```python
from build123d import *

# Parameters (mm, degrees)
EXTRUDE_1_DEPTH = 30


with BuildPart() as part:
    # 草图1 → 拉伸-薄壁1 (new body)
    with BuildSketch(Plane.XY):
        with BuildLine():
            Line((1246.5, -35.33), (-1246.5, -35.33))
            ThreePointArc((-1246.5, -35.33), (-1281.83, 0), (-1246.5, 35.33))
            Line((-1246.5, 35.33), (1246.5, 35.33))
            ThreePointArc((1246.5, 35.33), (1281.83, 0), (1246.5, -35.33))
        make_face()
        with BuildLine():
            Line((1246.5, -30.83), (-1246.5, -30.83))
            ThreePointArc((-1246.5, -30.83), (-1277.33, 0), (-1246.5, 30.83))
            Line((-1246.5, 30.83), (1246.5, 30.83))
            ThreePointArc((1246.5, 30.83), (1277.33, 0), (1246.5, -30.83))
        make_face(mode=Mode.SUBTRACT)
    extrude(amount=EXTRUDE_1_DEPTH)


solid = part.part
```
Design review of the part built by this model. Coordinates are the model's own, in mm. Coordinates: 2 decimals unless noted, no trailing zeros. Order: outer loops, then holes, each group sorted by start corner. A loop starts at its lowest first (then second) coordinate and runs counter-clockwise, first axis right, second up. Notation, with made-up numbers: (-2, -4.5) -> (13, -4.5) arc R22 cw to (13, 15.5) -> close; hole circle Ø3 at (-18.5, -38.5). An arc over 180 degrees is marked (long way). One line per item, written item: value. Start each with the question number.
Q1. Take a section at A-A, the plane y = 0. State the section outline as (x, z) points, then the cut area to 3 significant figures.
Q2. For probe 1 along X at (y, z) = (-2, 3.75); probe 2 along X at (y, z) = (3.5, 4.25); probe 3 along Y at (x, z) = (15, 7.5), list the stretches that pass through material, from the lowest coordinate up.
Q3. Take a section at C-C, the plane z = 10. State the section outline as (x, y) points.
Q4. Insertion check: pin 1 Ø6 at (y, z) = (5, 7) entering from -X; pin 2 Ø6 at (y, z) = (-5.5, 7.5) entering from +X. Each pin has a flat end and moves straight along its axis. Give the tip position at first contact, or say it passes through.
Q5. Take a section at B-B, the plane x = 747.5. State the section outline as (y, z) points, then the cut area to 3 significant figures.
Values follow:
1. outline: (-1281.83, 0) -> (-1277.33, 0) -> (-1277.33, 30) -> (-1281.83, 30) -> close; (1277.33, 0) -> (1281.83, 0) -> (1281.83, 30) -> (1277.33, 30) -> close
1. area: 270 mm2
2. probe 1: x = -1281.77 to -1277.27, 1277.27 to 1281.77
2. probe 2: x = -1281.66 to -1277.13, 1277.13 to 1281.66
2. probe 3: y = -35.33 to -30.83, 30.83 to 35.33
3. outline: (-1246.5, -35.33) -> (1246.5, -35.33) arc R35.33 ccw to (1246.5, 35.33) -> (-1246.5, 35.33) arc R35.33 ccw to start; hole (-1246.5, -30.83) -> (1246.5, -30.83) arc R30.83 ccw to (1246.5, 30.83) -> (-1246.5, 30.83) arc R30.83 ccw to start
4. pin 1: stops at x = -1281.77
4. pin 2: stops at x = 1281.74
5. outline: (-35.33, 0) -> (-30.83, 0) -> (-30.83, 30) -> (-35.33, 30) -> close; (30.83, 0) -> (35.33, 0) -> (35.33, 30) -> (30.83, 30) -> close
5. area: 270 mm2
